Verification items for the finished model (mm, model axes). A direction names the side the tool comes from. Round coordinates to 2 decimals unless told otherwise and drop trailing zeros. Write each loop counter-clockwise with the first axis right and the second up, starting at its lowest first coordinate (ties: lowest second). Pieces come first, ordered by that corner, then holes. Notation, with made-up numbers: (20, 6.25) - (44, 6.25) arc R37 ccw to (44, 45.25) - close; hole circle Ø7 at (4.5, -27). An arc over 180 degrees is marked (long way). Answer as a JSON object with one key per item and string values. Group by question number.
1) Section check C-C (y = -11). Enter the section's corners in (x, z).
2) Go/stop test with flat-tipped pins: pin 1 Ø6 at (y, z) = (12, -4) entering from -X; pin 2 Ø7 at (x, y) = (26.5, 11) entering from +Z; pin 3 Ø1.5 at (x, y) = (-63.5, -2.5) entering from -Z; pin 4 Ø5.5 at (x, z) = (-60.97, 0) entering from -Y. Record where each tip stops, or that it passes through.
3) Section check D-D (y = 11). Enter the section's corners in (x, z), then the cut area to 3 significant figures.
4) Mould release check, pull along Z, two halves, no side actions. Record for faces 6 (the flat face through (27, 0, 6)), 7 (the flat face through (-5.41, 14.63, 0.22)), 8 (the cylindrical face through (-15.012, 4.014, 0.55)): +Z half, -Z half, draft (parallel to the pull), parting line (faces both ways), or undercut.
5) Set-up check for faces 1 (the flat face through (-33, 3, 3)), 2 (the flat face through (26, 0, -6)), 3 (the cylindrical face through (-49.949, 37.286, 0.266)), 4 (the flat face through (-81.47, -5, 3)), 5 (the flat face through (16, 24, 0)): record each of +Z, -Z, +X, -X, +Y, -Y from which the full face is reachable in a straight line by a thin tool's end or side.
6) Section check B-B (z = 0). State how many separate pieces and enclosed holes the cut face has, then the cut area to 3 significant figures.
7) Section check A-A (x = 26.5). Enter the section's corners in (y, z).
8) Thickness scan on line 1 (Y direction, x = 26.5, z = -1.75); line 2 (X direction, y = -14, z = 24); line 3 (X direction, y = 14, z = 14). Record the ranges inside material, lowest first.
```python
from build123d import *

# Parameters (mm, degrees)
BASE_BLOCK_DEPTH           = 24
BASE_SLOT_SKETCH_R         = 3
BASE_SLOT_22X6_DEPTH       = 48
ANGLED_WEB_DEPTH           = 16
UPPER_BLOCK_SKETCH_R       = 20.5
UPPER_BLOCK_SKETCH_R_2     = 14
UPPER_BLOCK_DEPTH          = 19
SIDE_LUG_SKETCH_W          = 24
SIDE_LUG_SKETCH_H          = 16
SIDE_LUG_DEPTH             = 16
LUG_HOLE_SKETCH_R          = 3
LUG_HOLE_6_DEPTH           = 16
SPOT_FACE_RECESS_SKETCH_R  = 12.5
SPOT_FACE_RECESS_2MM_DEPTH = 2
SPOT_FACE_HOLE_SKETCH_R    = 6
SPOT_FACE_HOLE_12_DEPTH    = 96.223708731
VERTICAL_BORE_SKETCH_R     = 3
VERTICAL_BORE_CUT_DEPTH    = 50
PIVOT_HOUSING_DEPTH        = 40
TOP_PIN_HOLE_DEPTH         = 97.444568168
TOP_PIN_HOLE_DEPTH_BACK    = 97.444568168
TOP_PIN_HOLE_SKETCH_R      = 3
FRONT_PIN_HOLE_DEPTH       = 97.444568168
FRONT_PIN_HOLE_DEPTH_BACK  = 97.444568168
FRONT_PIN_HOLE_SKETCH_R    = 14
REAR_PAD_SKETCH_W          = 8.5
REAR_PAD_SKETCH_H          = 24
REAR_PAD_DEPTH             = 20
ANGLED_PAD_DEPTH           = 10
CONNECTING_RIB_DEPTH       = 10


with BuildPart() as part:
    # Base Block Sketch → Base Block (new, symmetric)
    with BuildSketch(Plane(origin=(0, 0, 0), x_dir=(1, 0, 0), z_dir=(0, 1, 0))):
        Polygon((0, -16), (0, 16), (12, 16), (12, 6), (41, 6), (41, -6), (12, -6), (12, -16), align=None)
    extrude(amount=BASE_BLOCK_DEPTH, both=True)

    # Base Slot Sketch → Base Slot 22x6 (cut)
    with BuildSketch(Plane.XY.offset(6)):
        with Locations((26.5, 11)):
            Circle(BASE_SLOT_SKETCH_R)
        with Locations(Location((26.5, -11, 0), (0, 0, 180))):
            Circle(BASE_SLOT_SKETCH_R)
    extrude(amount=-BASE_SLOT_22X6_DEPTH, mode=Mode.SUBTRACT)

    # Angled Web Sketch → Angled Web (add, symmetric)
    with BuildSketch(Plane.XY):
        Polygon((0, -24), (0, 24), (-10.969655115, 5), (-72.969655115, 5), (-72.969655115, -24), align=None)
    extrude(amount=ANGLED_WEB_DEPTH, both=True)

    # Upper Block Sketch → Upper Block (add, symmetric)
    with BuildSketch(Plane.XY):
        with Locations((-60.969655115, 20)):
            Circle(UPPER_BLOCK_SKETCH_R)
        with Locations((-60.969655115, 20)):
            Circle(UPPER_BLOCK_SKETCH_R_2, mode=Mode.SUBTRACT)
    extrude(amount=UPPER_BLOCK_DEPTH, both=True)

    # Side Lug Sketch → Side Lug (add)
    with BuildSketch(Plane.XZ.offset(24)):
        with Locations((-28, 24)):
            Rectangle(SIDE_LUG_SKETCH_W, SIDE_LUG_SKETCH_H)
        Polygon((-16, 16), (0, 16), (-16, 32), align=None)
    extrude(amount=-SIDE_LUG_DEPTH)

    # Lug Hole Sketch → Lug Hole Ø6 (cut)
    with BuildSketch(Plane(origin=(0, -8, 0), x_dir=(1, 0, 0), z_dir=(0, 1, 0))):
        with Locations(Location((-28.983060808, -24, 0), (0, 0, 270))):
            Circle(LUG_HOLE_SKETCH_R)
    extrude(amount=-LUG_HOLE_6_DEPTH, mode=Mode.SUBTRACT)

    # Spot Face Recess Sketch → Spot Face Recess 2mm (cut)
    with BuildSketch(Plane(origin=(0, 5, 0), x_dir=(1, 0, 0), z_dir=(0, 1, 0))):
        with Locations(Location((-27.5, 0, 0), (0, 0, 180))):
            Circle(SPOT_FACE_RECESS_SKETCH_R)
    extrude(amount=-SPOT_FACE_RECESS_2MM_DEPTH, mode=Mode.SUBTRACT)

    # Spot Face Hole Sketch → Spot Face Hole Ø12 (cut, through all)
    with BuildSketch(Plane(origin=(0, 3, 0), x_dir=(1, 0, 0), z_dir=(0, 1, 0))):
        with Locations(Location((-27.5, 0, 0), (0, 0, 180))):
            Circle(SPOT_FACE_HOLE_SKETCH_R)
    extrude(amount=-SPOT_FACE_HOLE_12_DEPTH, mode=Mode.SUBTRACT)

    # Vertical Bore Sketch → Vertical Bore Cut (cut)
    with BuildSketch(Plane(origin=(0, 0, 0), x_dir=(1, 0, 0), z_dir=(0, 1, 0))):
        with Locations(Location((-60.969655115, 0, 0), (0, 0, 90))):
            Circle(VERTICAL_BORE_SKETCH_R)
    extrude(amount=VERTICAL_BORE_CUT_DEPTH, mode=Mode.SUBTRACT)

    # Pivot Housing Sketch → Pivot Housing (add)
    with BuildSketch(Plane(origin=(0, 0, 0), x_dir=(1, 0, 0), z_dir=(0, 1, 0))):
        Polygon((-60.969655115, 0), (-60.969655115, 10), (-81.469655115, 10), (-81.469655115, -10), (-60.969655115, -10), align=None)
    extrude(amount=PIVOT_HOUSING_DEPTH)

    # Top Pin Hole Sketch → Top Pin Hole (cut, two sides: drawn at the far end of the back side and taken through both)
    with BuildSketch(Plane(origin=(0, 0, 0), x_dir=(1, 0, 0), z_dir=(0, 1, 0)).offset(-TOP_PIN_HOLE_DEPTH_BACK)):
        with Locations(Location((-60.969655115, 0, 0), (0, 0, 90))):
            Circle(TOP_PIN_HOLE_SKETCH_R)
    extrude(amount=TOP_PIN_HOLE_DEPTH + TOP_PIN_HOLE_DEPTH_BACK, mode=Mode.SUBTRACT)

    # Front Pin Hole Sketch → Front Pin Hole (cut, two sides: drawn at the far end of the back side and taken through both)
    with BuildSketch(Plane.XY.offset(-FRONT_PIN_HOLE_DEPTH_BACK)):
        with Locations((-60.969655115, 20)):
            Circle(FRONT_PIN_HOLE_SKETCH_R)
    extrude(amount=FRONT_PIN_HOLE_DEPTH + FRONT_PIN_HOLE_DEPTH_BACK, mode=Mode.SUBTRACT)

    # Rear Pad Sketch → Rear Pad (add)
    with BuildSketch(Plane.XY.offset(10)):
        with Locations((-77.219655115, -12)):
            Rectangle(REAR_PAD_SKETCH_W, REAR_PAD_SKETCH_H)
    extrude(amount=-REAR_PAD_DEPTH)

    # Angled Pad Sketch → Angled Pad (add, symmetric)
    with BuildSketch(Plane.XY):
        Polygon((-100.580876389, 20), (-100.580876389, 33), (-81.469655115, 33), (-81.469655115, 15.235037368), align=None)
    extrude(amount=ANGLED_PAD_DEPTH, both=True)

    # Connecting Rib Sketch → Connecting Rib (add)
    with BuildSketch(Plane.XY.offset(16)):
        with BuildLine():
            Line((-72.969655115, -24), (-81.469655115, -24))
            Line((-81.469655115, -24), (-81.469655115, 15.235037368))
            Line((-81.469655115, 15.235037368), (-80.90818894, 15.235037368))
            ThreePointArc((-80.90818894, 15.235037368), (-78.003666053, 8.594191332), (-72.969655115, 3.379229861))
            Line((-72.969655115, 3.379229861), (-72.969655115, -24))
        make_face()
    extrude(amount=-CONNECTING_RIB_DEPTH)


solid = part.part
```
Returned:
{
 "1": {"outline": "(-81.47, -10) - (-72.97, -10) - (-72.97, -16) - (12, -16) - (12, -6) - (23.5, -6) - (23.5, 6) - (12, 6) - (12, 16) - (0, 16) - (-16, 32) - (-40, 32) - (-40, 16) - (-81.47, 16) - close; (29.5, -6) - (41, -6) - (41, 6) - (29.5, 6) - close; hole circle Ø6 at (-60.97, 0); hole circle Ø12 at (-27.5, 0); hole circle Ø6 at (-28.98, 24)"},
 "2": {"pin 1": "x = -81.47", "pin 2": "z = 6", "pin 3": "z = -16", "pin 4": "through"},
 "3": {"outline": "(-81.47, -10) - (-79.39, -10) - (-79.39, -19) - (-71.69, -19) - (-71.69, 19) - (-79.39, 19) - (-79.39, 16) - (-81.47, 16) - close; (-50.25, -19) - (-42.55, -19) - (-42.55, 19) - (-50.25, 19) - close; (-7.51, -16) - (12, -16) - (12, -6) - (23.5, -6) - (23.5, 6) - (12, 6) - (12, 16) - (-7.51, 16) - close; (29.5, -6) - (41, -6) - (41, 6) - (29.5, 6) - close", "area": "1,540 mm2"},
 "4": {"face 6": "+Z half", "face 7": "draft", "face 8": "undercut"},
 "5": {"face 1": "+Y", "face 2": "-Z, +X, +Y, -Y", "face 3": "none", "face 4": "+Z, -Z, -X, -Y", "face 5": "+Z, -Z, +X, +Y"},
 "6": {"separate pieces": "3", "enclosed holes": "2", "area": "4,790 mm2"},
 "7": {"outline": "(-24, -6) - (-14, -6) - (-14, 6) - (-24, 6) - close; (-8, -6) - (8, -6) - (8, 6) - (-8, 6) - close; (14, -6) - (24, -6) - (24, 6) - (14, 6) - close"},
 "8": {"line 1": "-24 to -14, -8 to 8, 14 to 24", "line 2": "-40 to -31.98, -25.98 to -8", "line 3": "-81.47 to -73.62, -48.32 to -41.37, -5.77 to 12"}
}
